Part print with two shaded views. Sizes in mm from the minimum x, y, z corner. A direction names the side the tool comes from. Round coordinates to 2 decimals unless told otherwise and drop trailing zeros. Loops run counter-clockwise (first coordinate to the right, second up) from the corner with the lowest first, then second, coordinate; pieces in that order, holes last.
(1) Probe probe 1 along X at (y, z) = (1, 15); probe 2 along Y at (x, z) = (9.5, 25.25). List the from-to ranges inside material, lowest first.
(2) Tool access for the marked faces 1 and 2: list every direction of +Z, -Z, +X, -X, +Y, -Y with a clear straight run to the whole face (end or side of a thin tool).
(3) Cut at B-B on z = 15. List the corners of the cut face in (x, y).
(4) Cut at C-C on y = 2. List the corners of the cut face in (x, z).
(5) Flat gauge pins, fed straight in: pin 1 (7 mm diameter, centred on y = 22, z = 21.5, fed in from +X); pin 2 (11.5 mm diameter, centred on x = 22, z = 15, fed in from +Y). Where does each tip first touch, or does it go through?
(6) Cut at A-A on x = 22. List the corners of the cut face in (y, z).
(7) Cut at D-D on z = 7. List the corners of the cut face in (x, y).
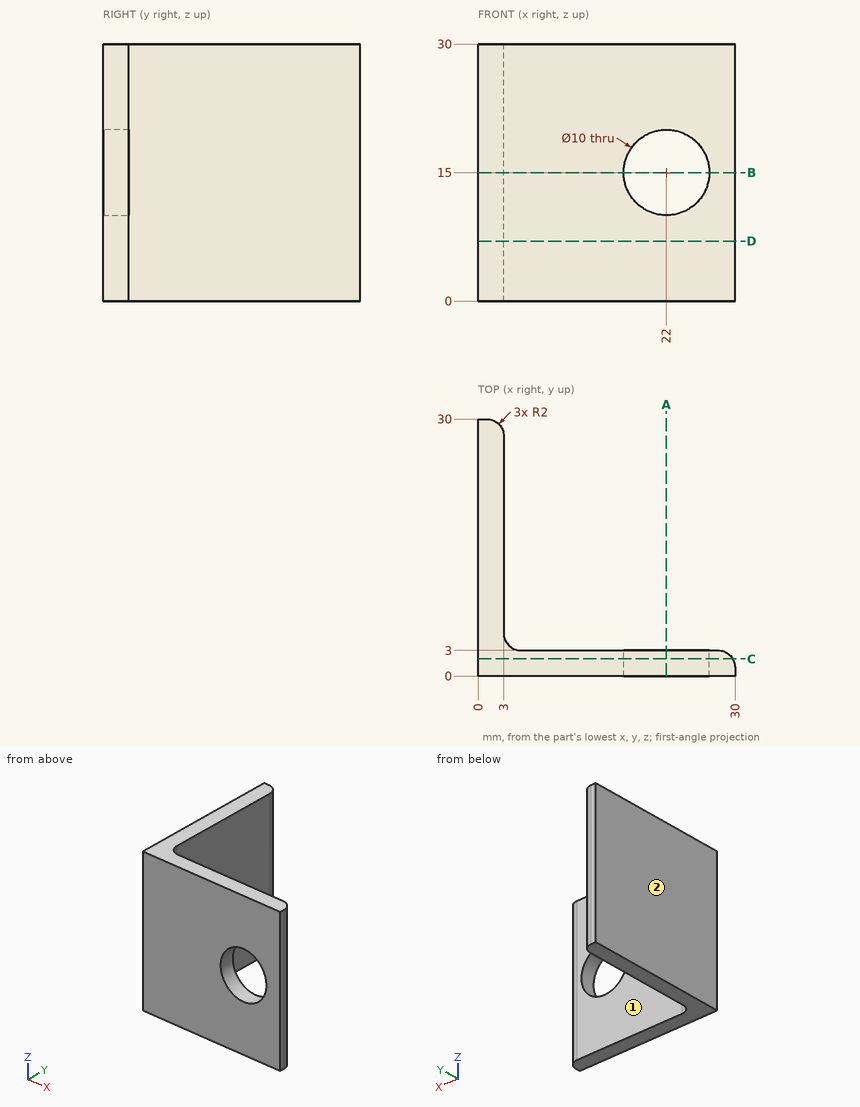
Final values:
1. probe 1: x = 0 to 17, 27 to 30
1. probe 2: y = 0 to 3
2. face 1: +Z, -Z, +X, +Y
2. face 2: +Z, -Z, -X, +Y, -Y
3. outline: (0, 0) - (17, 0) - (17, 3) - (5, 3) arc R2 cw to (3, 5) - (3, 28) arc R2 ccw to (1, 30) - (0, 30) - close; (27, 0) - (30, 0) - (30, 1) arc R2 ccw to (28, 3) - (27, 3) - close
4. outline: (0, 0) - (29.73, 0) - (29.73, 30) - (0, 30) - close; hole circle Ø10 at (22, 15)
5. pin 1: stops at x = 3
5. pin 2: stops at y = 3
6. outline: (0, 0) - (3, 0) - (3, 10) - (0, 10) - close; (0, 20) - (3, 20) - (3, 30) - (0, 30) - close
7. outline: (0, 0) - (30, 0) - (30, 1) arc R2 ccw to (28, 3) - (5, 3) arc R2 cw to (3, 5) - (3, 28) arc R2 ccw to (1, 30) - (0, 30) - close
